from build123d import *

# Parameters (mm, degrees)
EXTRUDE_364_DEPTH      = 7.5
SKETCH_4_W             = 0.6
SKETCH_4_H             = 11.392304845
CHAMFER_2049_SIZE      = 1.4
FILLET_2094_R          = 0.6
PATTERN_LINEAR_1_COUNT = 10
PATTERN_LINEAR_1_PITCH = 1.666666667


with BuildPart() as part:
    # 草图1 → Extrude 364 (new body)
    with BuildSketch(Plane(origin=(0, 0, 0), x_dir=(0, 0, -1), z_dir=(1, 0, 0))):
        Polygon((9, 5.196152423), (9, -5.196152423), (0, -10.392304845), (-9, -5.196152423), (-9, 5.196152423), (0, 10.392304845), align=None)
    extrude(amount=EXTRUDE_364_DEPTH)

    # 草图2 → 凸台-旋转1 (revolve)
    with BuildSketch(Plane.XY, mode=Mode.PRIVATE) as revolve_1_sk:
        Polygon((0, 0), (37.5, 0), (37.5, 4.4845), (37.5, 6), (7.791693541, 6), (0, 6), align=None)
    revolve(revolve_1_sk.sketch.rotate(Axis((0, 0, 0), (1, 0, 0)), 90), axis=Axis((0, 0, 0), (1, 0, 0)))

    # 草图3 → 切除-旋转1 (revolve, cut)
    with BuildSketch(Plane.XY):
        Polygon((0, 9), (3.690598923, 15.392304845), (3.690598923, 20.392304845), (-10, 20.392304845), (-10, 9), align=None)
    revolve(axis=Axis((0, 0, 0), (1, 0, 0)), mode=Mode.SUBTRACT)

    # 草图5 → 切除-旋转2 (revolve, cut)
    with BuildSketch(Plane.XY):
        Polygon((7.5, 9), (3.809401077, 15.392304845), (3.809401077, 20.392304845), (13.809401077, 20.392304845), (13.809401077, 9), align=None)
    revolve(axis=Axis((0, 0, 0), (1, 0, 0)), mode=Mode.SUBTRACT)

    # 草图4 → 切除-旋转3 (revolve, cut)
    with BuildSketch(Plane.XY, mode=Mode.PRIVATE) as cut_revolve_3_sk:
        with Locations((7.2, 14.696152423)):
            Rectangle(SKETCH_4_W, SKETCH_4_H)
    revolve(cut_revolve_3_sk.sketch.rotate(Axis((0, 0, 0), (1, 0, 0)), 270), axis=Axis((0, 0, 0), (1, 0, 0)), mode=Mode.SUBTRACT)

    # Chamfer 2049
    chamfer_2049_edges = [part.edges().sort_by_distance(p)[0] for p in [
        (37.5, 0, -6),
    ]]
    chamfer(chamfer_2049_edges, length=CHAMFER_2049_SIZE)

    # Fillet 2094
    fillet_2094_edges = [part.edges().sort_by_distance(p)[0] for p in [
        (7.5, 0, -6),
    ]]
    fillet(fillet_2094_edges, radius=FILLET_2094_R)

    # 草图6 → 切除-旋转4 (revolve, cut)
    with BuildSketch(Plane.XY):
        Polygon((22.5, -4.4845), (21.625025667, -6), (21.625025667, -7.5), (23.374974333, -7.5), (23.374974333, -6), align=None)
    cut_revolve_4 = revolve(axis=Axis((-3.175, 0, 0), (1, 0, 0)), mode=Mode.SUBTRACT)

    # 阵列(线性)1: 切除-旋转4 ×10
    with Locations(*[(i * PATTERN_LINEAR_1_PITCH, 0, 0) for i in range(1, PATTERN_LINEAR_1_COUNT)]):
        add(cut_revolve_4, mode=Mode.SUBTRACT)


solid = part.part
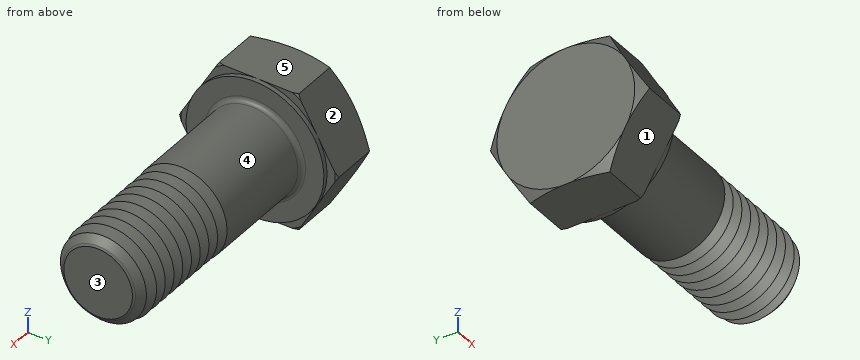
Could you check a few things on this model? Use its own coordinates, in mm. Face numbers are marked on the shaded views. A direction names the side the tool comes from. Coordinates: 2 decimals unless noted, no trailing zeros. Write each loop counter-clockwise with the first axis right and the second up, starting at its lowest first coordinate (ties: lowest second). Pieces come first, ordered by that corner, then holes. Notation, with made-up numbers: (33, 32) - (65, 32) arc R10 cw to (65, 49) - close; hole circle Ø6 at (25.5, 48.25). An arc over 180 degrees is marked (long way). Put each result on its own line as item: value. Start each with the question number.
Q1. I want a section at A-A on x = 18.5. Write out the boundary of the cut face in (y, z), plus the area to 3 significant figures.
Q2. Please list where these lines run through material, in increasing order: L1, parallel to X at y = 4.5, z = -7; L2, parallel to Z at x = 11, y = -3; L3, parallel to Y at x = 16.5, z = 4.25.
Q3. Thinking about a two-plate mould opening in Z: for the marked faces 1, 2 and 3, which applies, pulls with the +Z half, pulls with the -Z half, needs draft (parallel to the pull), parting line crosses it, or undercut?
Q4. Which directions (+Z, -Z, +X, -X, +Y, -Y) give clear straight access to the entire face, cutting with the end or side of a thin tool? Please do the marked faces 4 and 5.
Q5. I'm going to push flat-ended pins straight in: P1, Ø0.7, axis at y = 9, z = -2, coming from the +X side; P2, Ø1, axis at x = 33, y = -4.5, coming from the +Z side (3 decimals); P3, Ø3, axis at x = 21.5, z = 3.5, coming from the -Y side; P4, Ø3, axis at y = -6.5, z = -2, coming from the -X side. Where does each tip first touch, or does it pass through?
Checks:
1. outline: circle Ø12 at (0, 0)
1. area: 113 mm²
2. L1: 0 to 7.5
2. L2: -5.2 to 5.2
2. L3: -4.24 to 4.24
3. face 1: pulls with the -Z half
3. face 2: pulls with the +Z half
3. face 3: needs draft
4. face 4: +X
4. face 5: +Z, +X, -X, +Y, -Y
5. P1: x = 7.5
5. P2: z = 4.255
5. P3: y = -5.66
5. P4: x = 0
